Verification items for the finished model (mm, model axes). A direction names the side the tool comes from. Coordinates: 2 decimals unless noted, no trailing zeros. Order: outer loops, then holes, each group sorted by start corner. A loop starts at its lowest first (then second) coordinate and runs counter-clockwise, first axis right, second up. Notation, with made-up numbers: M -38.75,78 L -3.75,78 A19 ccw -3.75,91 Z; hole C 35.25,29.5 d7. An arc over 180 degrees is marked long. Answer as a JSON object with one key per item and string values. Group by question number.
(1) Material ranges on line 1 (X direction, y = -12.5, z = 0.25); line 2 (Y direction, x = -4.5, z = 3), recorded low to high.
(2) Gauge pin test, flat ends, axial feed: pin 1 Ø5 at (x, z) = (-10, 2.5) entering from -Y; pin 2 Ø6 at (y, z) = (-34, -3.5) entering from -X; pin 3 Ø3 at (x, z) = (-21, -2.5) entering from -Y. Record the tip position at first contact, or that the pin passes through.
(3) Cross-section at A-A (z = 0). Enter the section's corners in (x, y).
(4) Cross-section at C-C (y = -11). Enter the section's corners in (x, z).
(5) Cross-section at B-B (x = -16). Enter the section's corners in (y, z).
(6) Access from +Z, -Z, +X, -X, +Y, -Y to the whole of each face (thin tool, end or side, straight path). Record for faces 1 (the face through (-30, -60, 0)), 2 (the face through (-10.63, 4.88, 1.08)), 3 (the face through (-34.88, -34.84, 1.08)).
from build123d import *

# Parameters (mm, degrees)
SKETCH_2_R = 5
FILLET_1_R = 1


with BuildPart() as part:
    # 扫描1: sweep along a path in 草图1
    with BuildLine(Plane.XY) as sweep_1_path:
        Line((0, 0), (-20, 0))
        ThreePointArc((-20, 0), (-27.071067812, -2.928932188), (-30, -10))
        Line((-30, -10), (-30, -60))
    # 草图2 → 扫描1 (sweep)
    with BuildSketch(Plane(origin=(0, 0, 0), x_dir=(0, 0, -1), z_dir=(1, 0, 0))):
        Circle(SKETCH_2_R)
    sweep(path=sweep_1_path.line)

    # 圆角1
    fillet_1_edges = [part.edges().sort_by_distance(p)[0] for p in [
        (0, 0, 5),
        (-30, -60, 5),
    ]]
    fillet(fillet_1_edges, radius=FILLET_1_R)


solid = part.part
Taken from the geometry:
{
 "1": {"line 1": "x = -34.99 to -25.01", "line 2": "y = -4 to 4"},
 "2": {"pin 1": "stops at y = -5", "pin 2": "stops at x = -34.97", "pin 3": "stops at y = -5.22"},
 "3": {"outline": "M -35,-59 A1 ccw -34,-60 L -26,-60 A1 ccw -25,-59 L -25,-10 A5 cw -20,-5 L -1,-5 A1 ccw 0,-4 L 0,4 A1 ccw -1,5 L -20,5 A15 ccw -35,-10 Z"},
 "4": {"outline": "C -30,0 d10"},
 "5": {"outline": "C 0,0 d10"},
 "6": {"face 1": "+Z, -Z, +X, -X, -Y", "face 2": "+X", "face 3": "-Y"}
}
